The model under review builds one solid part; all positions refer to its coordinate system, in mm. A direction names the side the tool comes from. Coordinates: 2 decimals unless noted, no trailing zeros. Order: outer loops, then holes, each group sorted by start corner. A loop starts at its lowest first (then second) coordinate and runs counter-clockwise, first axis right, second up. Notation, with made-up numbers: M 31,-10.75 L 77,-10.75 A10 cw 77,4.25 Z; hole C 48.5,-5.75 d2. An arc over 180 degrees is marked long. Write each question's results on one line, items separated by ' | '.
from build123d import *


with BuildPart() as part:
    # Sketch1 → Revolve1 (revolve)
    with BuildSketch(Plane.XY, mode=Mode.PRIVATE) as revolve1_sk:
        Polygon((-2966.670374904, 0), (-2484.570374904, 0), (-2484.570374904, 10), (-2509.170378936, 10), (-2509.170378936, 17.25), (-2535.170378936, 17.25), (-2535.170378936, 10), (-2617.170378936, 10), (-2617.170378936, 21.4), (-2635.170378936, 21.4), (-2635.170378936, 10), (-2707.170253936, 10), (-2707.170253936, 21.55), (-2725.170253936, 21.55), (-2725.170253936, 10), (-2800.170132968, 10), (-2800.170132968, 21.7), (-2818.170132968, 21.7), (-2818.170132968, 10), (-2913.920034929, 10), (-2913.920034929, 21.85), (-2933.920034929, 21.85), (-2933.920034929, 10), (-2951.670374904, 10), (-2951.670374904, 25), (-2966.670374904, 25), align=None)
    revolve(revolve1_sk.sketch.rotate(Axis((-2966.670374904, 0, 0), (1, 0, 0)), 90), axis=Axis((-2966.670374904, 0, 0), (1, 0, 0)))


solid = part.part
1) Take a section at A-A on x = -2922. State the section outline as (y, z) points, plus the area to 3 significant figures.
Solutions:
outline: C 0,0 d43.7 | area: 1,500 mm2
2) For pin 1 (8 mm diameter, centred on x = -2806.5, z = 1, fed in from -Y); pin 2 (10 mm diameter, centred on x = -2632, y = 1, fed in from -Z); pin 3 (4 mm diameter, centred on x = -2707.5, z = -13.5, fed in from -Y), all flat-tipped, find the tip position at first contact; note any pin that passes through.
Solutions:
pin 1: y = -21.7 | pin 2: z = -21.4 | pin 3: y = -18.23
3) Take a section at B-B on x = -2837.5. State the section outline as (y, z) points.
Solutions:
outline: C 0,0 d20
4) For faces 1 (the flat face through (-2966.67, 0, 0)), 2 (the flat face through (-2617.17, 9.2, -4.5)), 3 (the cylindrical face through (-2716.296, -6.473, 20.555)), list the 3-axis set-ups (+Z, -Z, +X, -X, +Y, -Y) from which the entire face can be reached by the end or side of a thin tool; tool diameter is ignored.
Solutions:
face 1: +Z, -Z, -X, +Y, -Y | face 2: none | face 3: +X
5) To check wall thickness, follow line 1 along X through (y, z) = (-16, 3); line 2 along X through (y, z) = (6.5, -18); line 3 along Z through (x, y) = (-2818, 1). State the ranges of each line that lie inside material, in increasing order.
Solutions:
line 1: -2966.67 to -2951.67, -2933.92 to -2913.92, -2818.17 to -2800.17, -2725.17 to -2707.17, -2635.17 to -2617.17, -2535.17 to -2509.17 | line 2: -2966.67 to -2951.67, -2933.92 to -2913.92, -2818.17 to -2800.17, -2725.17 to -2707.17, -2635.17 to -2617.17 | line 3: -21.68 to 21.68
